from build123d import *

# Parameters (mm, degrees)
BORE_SKETCH_R      = 3.8
THROUGH_BORE_DEPTH = 22.354156504
RECESS_SKETCH_13_R = 6.5
RECESS_13X2_DEPTH  = 2


with BuildPart() as part:
    # Bush Profile Sketch → Bush Body (revolve)
    with BuildSketch(Plane.XY, mode=Mode.PRIVATE) as bush_body_sk:
        Polygon((0, 0), (0, 10), (3, 10), (16, 7), (16, 0), align=None)
    revolve(bush_body_sk.sketch.rotate(Axis((-1000, 0, 0), (1, 0, 0)), 90), axis=Axis((-1000, 0, 0), (1, 0, 0)))

    # Bore Sketch → Through Bore (cut, through all)
    with BuildSketch(Plane.ZY):
        Circle(BORE_SKETCH_R)
    extrude(amount=-THROUGH_BORE_DEPTH, mode=Mode.SUBTRACT)

    # Recess Sketch Ø13 → Recess Ø13x2 (cut)
    with BuildSketch(Plane.ZY):
        Circle(RECESS_SKETCH_13_R)
    extrude(amount=-RECESS_13X2_DEPTH, mode=Mode.SUBTRACT)


solid = part.part
Can you work these out from the model? Positions are in its coordinate system, mm. A direction names the side the tool comes from. Round coordinates to 2 decimals unless told otherwise and drop trailing zeros. Order: outer loops, then holes, each group sorted by start corner. A loop starts at its lowest first (then second) coordinate and runs counter-clockwise, first axis right, second up. Notation, with made-up numbers: M 13,89 L 43,89 A28 cw 43,107 Z; hole C 19,52 d3. An arc over 180 degrees is marked long. Use a Markdown table: item, result.
1) I'm going to push flat-ended pins straight in: P1, Ø6.5, axis at y = -3, z = -2.5, coming from the -X side; P2, Ø2, axis at x = 7, z = -3.5, coming from the -Y side; P3, Ø5, axis at x = 4, z = -5, coming from the +Y side; P4, Ø1.5, axis at x = 4.5, y = 3.5, coming from the +Z side. Where does each tip first touch, or does it pass through?
Geometry says:
| item | result |
|---|---|
| P1 | stops at x = 0 |
| P2 | stops at y = -8.81 |
| P3 | stops at y = 9.63 |
| P4 | stops at z = 9.32 |
2) If we mould it in two halves opening along Y, with no side actions, what happens to faces 1 (the face through (11.04, 7.95, -1.77)), 2 (the face through (8.902, 0.167, -3.796)), 3 (the face through (16, 3, 3)), 4 (the face through (0.986, -3.955, -5.158))? For each: +Y half, -Y half, draft (parallel to the pull), parting line (faces both ways), or undercut.
Geometry says:
| item | result |
|---|---|
| face 1 | parting line |
| face 2 | undercut |
| face 3 | draft |
| face 4 | undercut |
3) On a 3-axis mill with a long thin cutter (end or side, diameter ignored), from which of +Z, -Z, +X, -X, +Y, -Y can I reach the whole of each face in a straight line? I mean faces 5 (the face through (2, -3, 3)), 6 (the face through (2, 0, -10)). Say none if no direction works.
Geometry says:
| item | result |
|---|---|
| face 5 | -X |
| face 6 | +X, -X |
4) Imagine slicing it at A-A (z = 0). List the corners of the cut face in (x, y) for me.
Geometry says:
| item | result |
|---|---|
| outline | M 0,-10 L 3,-10 L 16,-7 L 16,-3.8 L 2,-3.8 L 2,-6.5 L 0,-6.5 Z; M 0,6.5 L 2,6.5 L 2,3.8 L 16,3.8 L 16,7 L 3,10 L 0,10 Z |
5) If I drill on line 1 along Y through (x, z) = (1.1, 0); line 2 along X through (y, z) = (-4, -5); line 3 along Z through (x, y) = (14.25, 0.5), over which ranges is the centre line in solid material (lowest first)?
Geometry says:
| item | result |
|---|---|
| line 1 | y = -10 to -6.5, 6.5 to 10 |
| line 2 | x = 2 to 16 |
| line 3 | z = -7.39 to -3.77, 3.77 to 7.39 |
